Can you work these out from the model? Positions are in its coordinate system, mm. A direction names the side the tool comes from. Give positions to 0.01 mm unless a question says otherwise; leave off trailing zeros. Write each loop counter-clockwise with the first axis right and the second up, starting at its lowest first coordinate (ties: lowest second). Pieces come first, ordered by that corner, then holes. Notation, with made-up numbers: (54, 48.5) - (71, 48.5) arc R33 ccw to (71, 79.5) - close; hole circle Ø4 at (85.5, 86.5). An arc over 180 degrees is marked (long way). Return JSON: item names as keys, results as strings. Group by question number.
from build123d import *

# Parameters (mm, degrees)
SKETCH1_R           = 9
BOSS_EXTRUDE1_DEPTH = 2
SKETCH2_R           = 7.5
BOSS_EXTRUDE2_DEPTH = 13
SKETCH3_R           = 7
BOSS_EXTRUDE3_DEPTH = 6
SKETCH5_R           = 5.75
BOSS_EXTRUDE4_DEPTH = 18
SKETCH4_R           = 4.75
CUT_EXTRUDE1_DEPTH  = 42.024382994
CHAMFER1_SIZE       = 0.5
CHAMFER2_SIZE       = 0.3
CHAMFER2_SIZE2      = 10


with BuildPart() as part:
    # Sketch1 → Boss-Extrude1 (new body)
    with BuildSketch(Plane.XY):
        Circle(SKETCH1_R)
    extrude(amount=BOSS_EXTRUDE1_DEPTH)

    # Sketch2 → Boss-Extrude2 (add)
    with BuildSketch(Plane.XY.offset(2)):
        with Locations(Location((0, 0, 0), (0, 0, 180))):
            Circle(SKETCH2_R)
    extrude(amount=BOSS_EXTRUDE2_DEPTH)

    # Sketch3 → Boss-Extrude3 (add)
    with BuildSketch(Plane.XY.offset(15)):
        Circle(SKETCH3_R)
    extrude(amount=BOSS_EXTRUDE3_DEPTH)

    # Sketch5 → Boss-Extrude4 (add)
    with BuildSketch(Plane.XY.offset(21)):
        Circle(SKETCH5_R)
    extrude(amount=BOSS_EXTRUDE4_DEPTH)

    # Sketch4 → Cut-Extrude1 (cut, through all)
    with BuildSketch(Plane(origin=(0, 0, 0), x_dir=(-1, 0, 0), z_dir=(0, 0, -1))):
        Circle(SKETCH4_R)
    extrude(amount=-CUT_EXTRUDE1_DEPTH, mode=Mode.SUBTRACT)

    # Chamfer1
    chamfer1_edges = [part.edges().sort_by_distance(p)[0] for p in [
        (-5.75, 0, 39),
    ]]
    chamfer(chamfer1_edges, length=CHAMFER1_SIZE)

    # Chamfer2
    chamfer2_edges = [part.edges().sort_by_distance(p)[0] for p in [
        (4.75, 0, 0),
    ]]
    chamfer2_side = [part.faces().sort_by_distance(p)[0] for p in [
        (-8.745441559, 0, 0),
    ]]
    chamfer(chamfer2_edges, length=CHAMFER2_SIZE, length2=CHAMFER2_SIZE2, reference=chamfer2_side[0])


solid = part.part
1) Imagine slicing it at A-A, the plane x = 0. Write out the boundary of the cut face in (y, z), and give its area (3 significant figures).
2) Imagine slicing it at C-C, the plane z = 32. Write out the boundary of the cut face in (x, y), and give its area (3 significant figures).
3) Will these pins go through, and if not, where does the flat tip stop? pin 1 Ø5 at (x, z) = (-0.5, 28) entering from +Y; pin 2 Ø1.5 at (y, z) = (3.5, 21) entering from -X; pin 3 Ø6 at (y, z) = (-3, 8) entering from -X.
4) I need wall thicknesses on line 1 along Y through (x, z) = (0, 16.75); line 2 along Y through (x, z) = (0, 26.75); line 3 along Z through (x, y) = (7.75, 2). Which ranges of each line are inside material? Lowest first, please.
5) On a 3-axis mill with a long thin cutter (end or side, diameter ignored), from which of +Z, -Z, +X, -X, +Y, -Y can I reach the whole of each face in a straight line? I mean faces 1 (the face through (4, -4, 0)), 2 (the face through (-1, 6, 21)), 3 (the face through (1.06, -4.78, 5.07)). Say none if no direction works.
6) We'd pull the mould along Y, two halves only. Please class faces 4 (the face through (2, 7, 15)), 5 (the face through (-0.75, 5.7, 29.63)), 6 (the face through (-2.192, -4.214, 24.297)): pulls with the +Y half, pulls with the -Y half, needs draft (parallel to the pull), parting line crosses it, or undercut.
7) Imagine slicing it at D-D, the plane x = -6.5. Write out the boundary of the cut face in (y, z), and give its area (3 significant figures).
Resolved:
{
 "1": {"outline": "(-9, 0) - (-5.05, 0) - (-4.75, 10) - (-4.75, 39) - (-5.25, 39) - (-5.75, 38.5) - (-5.75, 21) - (-7, 21) - (-7, 15) - (-7.5, 15) - (-7.5, 2) - (-9, 2) - close; (4.75, 10) - (5.05, 0) - (9, 0) - (9, 2) - (7.5, 2) - (7.5, 15) - (7, 15) - (7, 21) - (5.75, 21) - (5.75, 38.5) - (5.25, 39) - (4.75, 39) - close", "area": "148 mm^2"},
 "2": {"outline": "circle Ø11.5 at (0, 0); hole circle Ø9.5 at (0, 0)", "area": "33.0 mm^2"},
 "3": {"pin 1": "y = 5.75", "pin 2": "x = -6.44", "pin 3": "x = -7.5"},
 "4": {"line 1": "-7 to -4.75, 4.75 to 7", "line 2": "-5.75 to -4.75, 4.75 to 5.75", "line 3": "0 to 2"},
 "5": {"face 1": "-Z, +X, -X, +Y, -Y", "face 2": "+Z", "face 3": "-Z"},
 "6": {"face 4": "needs draft", "face 5": "parting line crosses it", "face 6": "undercut"},
 "7": {"outline": "(-6.22, 0) - (6.22, 0) - (6.22, 2) - (3.74, 2) - (3.74, 15) - (2.6, 15) - (2.6, 21) - (-2.6, 21) - (-2.6, 15) - (-3.74, 15) - (-3.74, 2) - (-6.22, 2) - close", "area": "153 mm^2"}
}
